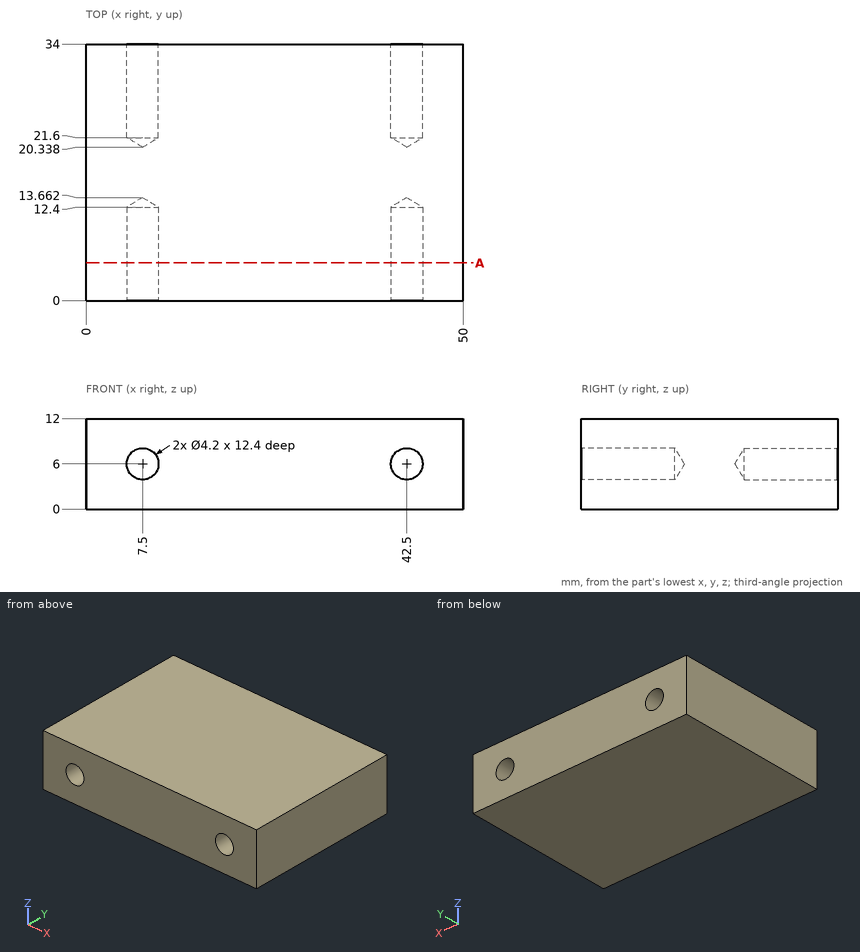
Here's the drawing with two shaded views (mm, measured from the low corner). I have some questions. Coordinates: 2 decimals unless noted, no trailing zeros. Loops run counter-clockwise (first coordinate to the right, second up) from the corner with the lowest first, then second, coordinate; pieces in that order, holes last. Notation, with made-up numbers: (-39, 8) -> (-18, 8) arc R10 ccw to (-18, 24) -> close; hole circle Ø10 at (-19, 84). An arc over 180 degrees is marked (long way). Answer in a Markdown table with one row per item.
(1) Imagine slicing it at A-A (y = 5). List the corners of the cut face in (x, z) for me, plus the area to 3 significant figures.
Results found:
| item | result |
|---|---|
| outline | (0, 0) -> (50, 0) -> (50, 12) -> (0, 12) -> close; hole circle Ø4.2 at (7.5, 6); hole circle Ø4.2 at (42.5, 6) |
| area | 572 mm^2 |
(2) Will these pins go through, and if not, where does the flat tip stop? pin 1 Ø3.5 at (x, z) = (42.5, 6) entering from +Y; pin 2 Ø3.5 at (x, z) = (7.5, 6) entering from -Y.
Results found:
| item | result |
|---|---|
| pin 1 | stops at y = 21.39 |
| pin 2 | stops at y = 12.61 |
(3) If I drill on probe 1 along X at (y, z) = (26.5, 6); probe 2 along Z at (x, y) = (7.5, 29.75); probe 3 along X at (y, z) = (8.5, 7.25), over which ranges is the centre line in solid material (lowest first)?
Results found:
| item | result |
|---|---|
| probe 1 | x = 0 to 5.4, 9.6 to 40.4, 44.6 to 50 |
| probe 2 | z = 0 to 3.9, 8.1 to 12 |
| probe 3 | x = 0 to 5.81, 9.19 to 40.81, 44.19 to 50 |
